```python
from build123d import *

# Parameters (mm, degrees)
BOSS_EXTRUDE1_DEPTH = 130
CHAMFER1_SIZE       = 5
SKETCH2_R           = 24.15
CUT_EXTRUDE1_DEPTH  = 130
CUT_EXTRUDE2_DEPTH  = 130


with BuildPart() as part:
    # Sketch1 → Boss-Extrude1 (new body)
    with BuildSketch(Plane.XY):
        with BuildLine():
            Line((0, 0), (0, -25.5))
            ThreePointArc((0, -25.5), (1.318019485, -28.681980515), (4.5, -30))
            Line((4.5, -30), (35.5, -30))
            ThreePointArc((35.5, -30), (38.681980515, -28.681980515), (40, -25.5))
            Line((40, -25.5), (40, 0))
            Line((40, 0), (37, 0))
            Line((37, 0), (37, -25.5))
            ThreePointArc((37, -25.5), (36.560660172, -26.560660172), (35.5, -27))
            Line((35.5, -27), (4.5, -27))
            ThreePointArc((4.5, -27), (3.439339828, -26.560660172), (3, -25.5))
            Line((3, -25.5), (3, 0))
            Line((3, 0), (0, 0))
        make_face()
    extrude(amount=BOSS_EXTRUDE1_DEPTH)

    # Chamfer1
    chamfer1_edges = [part.edges().sort_by_distance(p)[0] for p in [
        (38.5, 0, 0),
        (1.5, 0, 0),
    ]]
    chamfer(chamfer1_edges, length=CHAMFER1_SIZE)

    # Sketch2 → Cut-Extrude1 (cut)
    with BuildSketch(Plane(origin=(40, 0, 0), x_dir=(0, 0, -1), z_dir=(1, 0, 0))):
        with Locations((-149.15, -12.75)):
            Circle(SKETCH2_R)
    extrude(amount=-CUT_EXTRUDE1_DEPTH, mode=Mode.SUBTRACT)

    # Sketch3 → Cut-Extrude2 (cut)
    with BuildSketch(Plane.XZ.offset(30)):
        with BuildLine():
            Line((24.5, 96), (24.5, 21))
            ThreePointArc((24.5, 21), (20, 16.5), (15.5, 21))
            Line((15.5, 21), (15.5, 96))
            ThreePointArc((15.5, 96), (20, 100.5), (24.5, 96))
        make_face()
    extrude(amount=-CUT_EXTRUDE2_DEPTH, mode=Mode.SUBTRACT)


solid = part.part
```
Geometry check sheet. Reference: the model listing, model coordinates, mm. A direction names the side the tool comes from. Coordinates: 2 decimals unless noted, no trailing zeros. Loops run counter-clockwise (first coordinate to the right, second up) from the corner with the lowest first, then second, coordinate; pieces in that order, holes last. Notation, with made-up numbers: (32.5, 69) - (72.5, 69) arc R3 ccw to (72.5, 73) - close; hole circle Ø8 at (35, 7.5). An arc over 180 degrees is marked (long way). One line per item, written item: value. Start each with the question number.
(1) Cross-section at C-C on y = -15. Enter the section's corners in (x, z), plus the area to 3 significant figures.
(2) Cross-section at B-B on x = 20. Enter the section's corners in (y, z).
(3) Tool access check on faces 1 (the cylindrical face through (1.283, -28.647, 64.09)), 2 (the flat face through (24.5, -29, 59)), 3 (the flat face through (27, -27, 64)). Record the directions out of +Z, -Z, +X, -X, +Y, -Y that give a thin tool (end or side, any length) a straight path to the whole face; none if there is none.
(4) Depth check by flat-ended pin: P1, Ø9.5, axis at x = 27.5, z = 77, coming from the +Y side; P2, Ø1.5, axis at y = -29, z = 47, coming from the -X side; P3, Ø1.5, axis at y = -29, z = 57, coming from the +X side. Enter the tip coordinate at first touch or a pass-through.
(5) Mould release check, pull along Z, two halves, no side actions. Record for faces 4 (the flat face through (15.5, -29, 58)), 5 (the flat face through (20, -29, 130)), 6 (the flat face through (39, -3, 2)), 7 (the flat face through (37, -13, 63)): released by +Z, released by -Z, zero draft, split by the parting line, or undercut.
(6) Cross-section at A-A on z = 40.5. Enter the section's corners in (x, y), plus the area to 3 significant figures.
(7) Material ranges on line 1 (X direction, y = -18.5, z = 48); line 2 (Y direction, x = 10, z = 47); line 3 (Y direction, x = 36.5, z = 98), recorded low to high. Write a range as [from, to].
(8) Cross-section at D-D on z = 110.5. Enter the section's corners in (x, y), plus the area to 3 significant figures.
Results below:
1. outline: (0, 0) - (3, 0) - (3, 125.11) - (0, 125.11) - close; (37, 0) - (40, 0) - (40, 125.11) - (37, 125.11) - close
1. area: 751 mm2
2. outline: (-30, 0) - (-27, 0) - (-27, 16.5) - (-30, 16.5) - close; (-30, 100.5) - (-27, 100.5) - (-27, 129.65) arc R24.15 cw to (-27.46, 130) - (-30, 130) - close
3. face 1: +Z, -Z, -X, -Y
3. face 2: +Y, -Y
3. face 3: +Z, -Z, +Y
4. P1: stops at y = -27
4. P2: stops at x = 0.94
4. P3: stops at x = 39.06
5. face 4: undercut
5. face 5: released by +Z
5. face 6: released by -Z
5. face 7: zero draft
6. outline: (0, -25.5) arc R4.5 ccw to (4.5, -30) - (15.5, -30) - (15.5, -27) - (4.5, -27) arc R1.5 cw to (3, -25.5) - (3, 0) - (0, 0) - close; (24.5, -30) - (35.5, -30) arc R4.5 ccw to (40, -25.5) - (40, 0) - (37, 0) - (37, -25.5) arc R1.5 cw to (35.5, -27) - (24.5, -27) - close
6. area: 247 mm2
7. line 1: x = [0, 3], [37, 40]
7. line 2: y = [-30, -27]
7. line 3: y = [-29.89, -26.62]
8. outline: (0, -25.5) arc R4.5 ccw to (4.5, -30) - (35.5, -30) arc R4.5 ccw to (40, -25.5) - (40, 0) - (37, 0) - (37, -25.5) arc R1.5 cw to (35.5, -27) - (4.5, -27) arc R1.5 cw to (3, -25.5) - (3, 0) - (0, 0) - close
8. area: 274 mm2
